Input: part model. Units: mm. Frame: model coordinates. Coordinates: 2 decimals unless noted, no trailing zeros. Loops run counter-clockwise (first coordinate to the right, second up) from the corner with the lowest first, then second, coordinate; pieces in that order, holes last.
```python
from build123d import *

# Parameters (mm, degrees)
EXTRUDE_1_DEPTH = 734


with BuildPart() as part:
    # 草图2 → 拉伸-薄壁1 (new, symmetric)
    with BuildSketch(Plane.XY):
        with BuildLine():
            Line((-11, 15), (11, 15))
            ThreePointArc((11, 15), (13.828427125, 13.828427125), (15, 11))
            Line((15, 11), (15, -11))
            ThreePointArc((15, -11), (13.828427125, -13.828427125), (11, -15))
            Line((11, -15), (-11, -15))
            ThreePointArc((-11, -15), (-13.828427125, -13.828427125), (-15, -11))
            Line((-15, -11), (-15, 11))
            ThreePointArc((-15, 11), (-13.828427125, 13.828427125), (-11, 15))
        make_face()
        with BuildLine():
            Line((-11, 12), (11, 12))
            ThreePointArc((11, 12), (11.707106781, 11.707106781), (12, 11))
            Line((12, 11), (12, -11))
            ThreePointArc((12, -11), (11.707106781, -11.707106781), (11, -12))
            Line((11, -12), (-11, -12))
            ThreePointArc((-11, -12), (-11.707106781, -11.707106781), (-12, -11))
            Line((-12, -11), (-12, 11))
            ThreePointArc((-12, 11), (-11.707106781, 11.707106781), (-11, 12))
        make_face(mode=Mode.SUBTRACT)
    extrude(amount=EXTRUDE_1_DEPTH, both=True)


solid = part.part
```
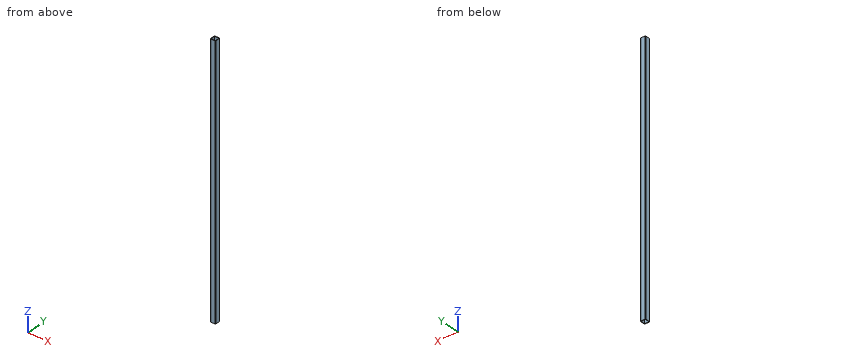
Item 1: Line query: L1, parallel to X at y = 4.75, z = -61.5; L2, parallel to Y at x = -13.25, z = -389. Output: solid intervals per line, ascending.
Result:
L1: x = -15 to -12, 12 to 15
L2: y = -14.31 to 14.31
Item 2: Section query C-C (z = 268). Output: boundary loops of the cut face in (x, y), then the cut area to 3 significant figures.
Result:
outline: (-15, -11) arc R4 ccw to (-11, -15) - (11, -15) arc R4 ccw to (15, -11) - (15, 11) arc R4 ccw to (11, 15) - (-11, 15) arc R4 ccw to (-15, 11) - close; hole (-12, -11) arc R1 ccw to (-11, -12) - (11, -12) arc R1 ccw to (12, -11) - (12, 11) arc R1 ccw to (11, 12) - (-11, 12) arc R1 ccw to (-12, 11) - close
area: 311 mm2
Item 3: Section query A-A (y = 2.25). Output: boundary loops of the cut face in (x, z), then the cut area to 3 significant figures.
Result:
outline: (-15, -734) - (-12, -734) - (-12, 734) - (-15, 734) - close; (12, -734) - (15, -734) - (15, 734) - (12, 734) - close
area: 8,810 mm2
